Geometry check sheet. Reference: the model listing, model coordinates, mm. A direction names the side the tool comes from. Give positions to 0.01 mm unless a question says otherwise; leave off trailing zeros. Order: outer loops, then holes, each group sorted by start corner. A loop starts at its lowest first (then second) coordinate and runs counter-clockwise, first axis right, second up. Notation, with made-up numbers: M 12.5,83 L 69.5,83 A22 ccw 69.5,95 Z; hole C 72.25,22.5 d2. An arc over 180 degrees is marked long. Answer as CSV lines item,"result". Start each with the question number.
Q1. Section check D-D, the plane x = 35. Record the boundary of the cut face in (y, z), then the cut area to 3 significant figures.
Q2. Section check A-A, the plane y = 6. Record the boundary of the cut face in (x, z), then the cut area to 3 significant figures.
Q3. Section check C-C, the plane y = 17. Record the boundary of the cut face in (x, z).
Q4. Go/stop test with flat-tipped pins: pin 1 (4.5 mm diameter, centred on x = 50, z = 15, fed in from +Y); pin 2 (11.5 mm diameter, centred on x = -25, y = 4.5, fed in from +Z); pin 3 (12 mm diameter, centred on x = 22.5, z = -8.5, fed in from +Y); pin 4 (6 mm diameter, centred on x = -24.5, y = 54, fed in from -Z). Record where each tip stops, or that it passes through.
Q5. Section check B-B, the plane x = 54.5. Record the boundary of the cut face in (y, z).
Q6. Mould release check, pull along Z, two halves, no side actions. Record for faces 1 (the cylindrical face through (-15.62, 35.62, -3.47)), 2 (the flat face through (22.322, 40.611, -19.382)), 3 (the flat face through (-0.1, 52.95, 18.2)), 4 (the cylindrical face through (-29.774, 5.197, -27.077)): +Z half, -Z half, draft (parallel to the pull), parting line (faces both ways), or undercut.
Q7. Set-up check for faces 5 (the flat face through (40, 31, -19)), 6 (the flat face through (-24, 5, 36)), 7 (the cylindrical face through (51.785, 40.235, -15.234)), 8 (the flat face through (40, 31, 19)): record each of +Z, -Z, +X, -X, +Y, -Y from which the full face is reachable in a straight line by a thin tool's end or side.
Q8. Thickness scan on line 1 (X direction, y = 43, z = 6.5); line 2 (X direction, y = 39, z = 0); line 3 (X direction, y = 24, z = 0). Record the ranges inside material, lowest first.
```python
from build123d import *

# Parameters (mm, degrees)
BASE_FLANGE_DEPTH                 = 10.25
TAPERED_COLUMN_SKETCH_R           = 35
TAPERED_COLUMN_DEPTH              = 42.7
TAPERED_COLUMN_TAPER              = 18.65
TOP_BOSS_SKETCH_R                 = 18
TOP_BOSS_DEPTH                    = 15.3
TOP_COLLAR_SKETCH_R               = 18
TOP_COLLAR_45DEG_TAPER_DEPTH      = 2
TOP_COLLAR_45DEG_TAPER_TAPER      = 45
SIDE_BOSS_DEPTH                   = 42.45
SIDE_BOSS_HOLES_SKETCH_R          = 2
SIDE_BOSS_HOLES_4X_DEPTH_10_DEPTH = 10
SECONDARY_HOLES_SKETCH_R          = 1.8
SECONDARY_HOLES_4X_DEPTH_5_DEPTH  = 5
SIDE_BORE_SKETCH_R                = 12
SIDE_BORE_DEPTH                   = 177
MAIN_BORE_SKETCH_R                = 16
MAIN_BORE_DEPTH                   = 177
FLANGE_HOLES_SKETCH_R             = 2
FLANGE_HOLES_4X_DEPTH             = 177


with BuildPart() as part:
    # Base Flange Sketch → Base Flange (new body)
    with BuildSketch(Plane(origin=(0, 0, 0), x_dir=(1, 0, 0), z_dir=(0, 1, 0))):
        with BuildLine():
            Line((58.058170092, 17.206565455), (40.981411355, 28.048001668))
            ThreePointArc((40.981411355, 28.048001668), (39.953813512, 28.512142384), (38.837512739, 28.671065375))
            Line((38.837512739, 28.671065375), (27.817939746, 28.671065375))
            ThreePointArc((27.817939746, 28.671065375), (26.436324443, 28.917248763), (25.224774509, 29.625495798))
            ThreePointArc((25.224774509, 29.625495798), (6.486223775, 38.365194531), (-14.083923128, 36.271233224))
            ThreePointArc((-14.083923128, 36.271233224), (-14.795259826, 36.068393006), (-15.531783042, 36))
            Line((-15.531783042, 36), (-28, 36))
            Line((-28, 36), (-32.472135955, 36))
            ThreePointArc((-32.472135955, 36), (-34.105129117, 35.651483717), (-35.453559925, 34.666666667))
            ThreePointArc((-35.453559925, 34.666666667), (-37.34172359, 31.568220898), (-38, 28))
            Line((-38, 28), (-38, 8.364164649))
            ThreePointArc((-38, 8.364164649), (-38.909629274, 0), (-38, -8.364164649))
            Line((-38, -8.364164649), (-38, -28))
            ThreePointArc((-38, -28), (-37.34172359, -31.568220898), (-35.453559925, -34.666666667))
            ThreePointArc((-35.453559925, -34.666666667), (-34.105129117, -35.651483717), (-32.472135955, -36))
            Line((-32.472135955, -36), (-28, -36))
            Line((-28, -36), (-15.531783042, -36))
            ThreePointArc((-15.531783042, -36), (-14.795259826, -36.068393006), (-14.083923128, -36.271233224))
            ThreePointArc((-14.083923128, -36.271233224), (6.486223775, -38.365194531), (25.224774509, -29.625495798))
            ThreePointArc((25.224774509, -29.625495798), (26.436324443, -28.917248763), (27.817939746, -28.671065375))
            Line((27.817939746, -28.671065375), (38.837512739, -28.671065375))
            ThreePointArc((38.837512739, -28.671065375), (39.953813512, -28.512142384), (40.981411355, -28.048001668))
            Line((40.981411355, -28.048001668), (58.058170092, -17.206565455))
            ThreePointArc((58.058170092, -17.206565455), (69, 0), (58.058170092, 17.206565455))
        make_face()
    extrude(amount=BASE_FLANGE_DEPTH)

    # Tapered Column Sketch → Tapered Column (add)
    with BuildSketch(Plane(origin=(0, 10.25, 0), x_dir=(1, 0, 0), z_dir=(0, 1, 0))):
        Circle(TAPERED_COLUMN_SKETCH_R)
    extrude(amount=TAPERED_COLUMN_DEPTH, taper=TAPERED_COLUMN_TAPER)

    # Top Boss Sketch → Top Boss (add)
    with BuildSketch(Plane(origin=(0, 52.95, 0), x_dir=(1, 0, 0), z_dir=(0, 1, 0))):
        with Locations(Location((0, 0, 0), (0, 0, 270))):
            Circle(TOP_BOSS_SKETCH_R)
    extrude(amount=TOP_BOSS_DEPTH)

    # Top Collar Sketch → Top Collar 45deg Taper (add)
    with BuildSketch(Plane(origin=(0, 68.25, 0), x_dir=(1, 0, 0), z_dir=(0, 1, 0))):
        with Locations(Location((0, 0, 0), (0, 0, 270))):
            Circle(TOP_COLLAR_SKETCH_R)
    extrude(amount=TOP_COLLAR_45DEG_TAPER_DEPTH, taper=TOP_COLLAR_45DEG_TAPER_TAPER)

    # Side Boss Sketch → Side Boss (add)
    with BuildSketch(Plane(origin=(0, 10.25, 0), x_dir=(1, 0, 0), z_dir=(0, 1, 0))):
        with BuildLine():
            ThreePointArc((50, -19), (69, 0), (50, 19))
            Line((50, 19), (29.393876913, 19))
            Line((29.393876913, 19), (2.218603036, 20.468479678))
            ThreePointArc((2.218603036, 20.468479678), (20.588367098, 0), (2.218603036, -20.468479678))
            Line((2.218603036, -20.468479678), (29.393876913, -19))
            Line((29.393876913, -19), (50, -19))
        make_face()
    extrude(amount=SIDE_BOSS_DEPTH)

    # Side Boss Holes Sketch → Side Boss Holes 4x Depth 10 (cut)
    with BuildSketch(Plane(origin=(0, 52.7, 0), x_dir=(1, 0, 0), z_dir=(0, 1, 0))):
        with Locations(Location((35, 0, 0), (0, 0, 270))):
            Circle(SIDE_BOSS_HOLES_SKETCH_R)
        with Locations(Location((50, 15, 0), (0, 0, 270))):
            Circle(SIDE_BOSS_HOLES_SKETCH_R)
        with Locations(Location((65, 0, 0), (0, 0, 270))):
            Circle(SIDE_BOSS_HOLES_SKETCH_R)
        with Locations(Location((50, -15, 0), (0, 0, 270))):
            Circle(SIDE_BOSS_HOLES_SKETCH_R)
    extrude(amount=-SIDE_BOSS_HOLES_4X_DEPTH_10_DEPTH, mode=Mode.SUBTRACT)

    # Secondary Holes Sketch → Secondary Holes 4x Depth 5 (cut)
    with BuildSketch(Plane(origin=(0, 42.7, 0), x_dir=(1, 0, 0), z_dir=(0, 1, 0))):
        with Locations(Location((35, 0, 0), (0, 0, 270))):
            Circle(SECONDARY_HOLES_SKETCH_R)
        with Locations(Location((65, 0, 0), (0, 0, 270))):
            Circle(SECONDARY_HOLES_SKETCH_R)
        with Locations(Location((50, -15, 0), (0, 0, 270))):
            Circle(SECONDARY_HOLES_SKETCH_R)
        with Locations(Location((50, 15, 0), (0, 0, 270))):
            Circle(SECONDARY_HOLES_SKETCH_R)
    extrude(amount=-SECONDARY_HOLES_4X_DEPTH_5_DEPTH, mode=Mode.SUBTRACT)

    # Side Bore Sketch → Side Bore (cut)
    with BuildSketch(Plane(origin=(0, 52.7, 0), x_dir=(1, 0, 0), z_dir=(0, 1, 0))):
        with Locations(Location((50, 0, 0), (0, 0, 270))):
            Circle(SIDE_BORE_SKETCH_R)
    extrude(amount=-SIDE_BORE_DEPTH, mode=Mode.SUBTRACT)

    # Main Bore Sketch → Main Bore (cut)
    with BuildSketch(Plane(origin=(0, 70.25, 0), x_dir=(1, 0, 0), z_dir=(0, 1, 0))):
        with Locations(Location((0, 0, 0), (0, 0, 270))):
            Circle(MAIN_BORE_SKETCH_R)
    extrude(amount=-MAIN_BORE_DEPTH, mode=Mode.SUBTRACT)

    # Flange Holes Sketch → Flange Holes 4x (cut)
    with BuildSketch(Plane(origin=(0, 10.25, 0), x_dir=(1, 0, 0), z_dir=(0, 1, 0))):
        with Locations(Location((40, -24, 0), (0, 0, 270))):
            Circle(FLANGE_HOLES_SKETCH_R)
        with Locations(Location((40, 24, 0), (0, 0, 270))):
            Circle(FLANGE_HOLES_SKETCH_R)
        with Locations(Location((-28, 28, 0), (0, 0, 270))):
            Circle(FLANGE_HOLES_SKETCH_R)
        with Locations(Location((-28, -28, 0), (0, 0, 270))):
            Circle(FLANGE_HOLES_SKETCH_R)
    extrude(amount=-FLANGE_HOLES_4X_DEPTH, mode=Mode.SUBTRACT)


solid = part.part
```
Answer block:
1,outline,"M 0,-28.67 L 10.25,-28.67 L 10.25,-19 L 52.7,-19 L 52.7,-2 L 42.7,-2 L 42.7,-1.8 L 37.7,-1.8 L 37.7,1.8 L 42.7,1.8 L 42.7,2 L 52.7,2 L 52.7,19 L 10.25,19 L 10.25,28.67 L 0,28.67 Z"
1,area,"2,140 mm2"
2,outline,"M -38,-28 A10 ccw -35.45,-34.67 A4 ccw -32.47,-36 L -15.53,-36 A4 cw -14.08,-36.27 A38.91 ccw 25.22,-29.63 A4 cw 27.82,-28.67 L 38.84,-28.67 A4 ccw 40.98,-28.05 L 58.06,-17.21 A19 ccw 58.06,17.21 L 40.98,28.05 A4 ccw 38.84,28.67 L 27.82,28.67 A4 cw 25.22,29.63 A38.91 ccw -14.08,36.27 A4 cw -15.53,36 L -32.47,36 A4 ccw -35.45,34.67 A10 ccw -38,28 L -38,8.36 A38.91 ccw -38,-8.36 Z; hole C -28,-28 d4; hole C -28,28 d4; hole C 0,0 d32; hole C 40,-24 d4; hole C 50,0 d24; hole C 40,24 d4"
2,area,"5,240 mm2"
3,outline,"M 26.53,-19.15 L 29.39,-19 L 50,-19 A19 ccw 50,19 L 29.39,19 L 26.53,19.15 A32.72 ccw long Z; hole C 0,0 d32; hole C 50,0 d24"
4,pin 1,"stops at y = 52.7"
4,pin 2,"stops at z = 36"
4,pin 3,"stops at y = 52.95"
4,pin 4,"passes through"
5,outline,"M 0,-19.47 L 10.25,-19.47 L 10.25,-18.46 L 52.7,-18.46 L 52.7,-11.12 L 0,-11.12 Z; M 0,11.12 L 52.7,11.12 L 52.7,18.46 L 10.25,18.46 L 10.25,19.47 L 0,19.47 Z"
6,face 1,"undercut"
6,face 2,"-Z half"
6,face 3,"draft"
6,face 4,"undercut"
7,face 5,"-Z, +X, +Y"
7,face 6,"+Z, -X, +Y, -Y"
7,face 7,"+Y"
7,face 8,"+Z, +X, +Y"
8,line 1,"x = -23.05 to -14.62, 14.62 to 39.91, 60.09 to 67.85"
8,line 2,"x = -25.3 to -16, 16 to 33.2, 36.8 to 38, 62 to 63.2, 66.8 to 69"
8,line 3,"x = -30.36 to -16, 16 to 38, 62 to 69"
